from build123d import *

# Parameters (mm, degrees)
SKETCH1_W           = 71.75
SKETCH1_H           = 71.75
SKETCH1_R           = 4
BOSS_EXTRUDE1_DEPTH = 10
FILLET1_R           = 5
FILLET2_R           = 1
FILLET4_R           = 0.15
SKETCH2_R           = 1.525
CUT_EXTRUDE1_DEPTH  = 10


with BuildPart() as part:
    # Sketch1 → Boss-Extrude1 (new body)
    with BuildSketch(Plane.XY):
        Rectangle(SKETCH1_W, SKETCH1_H)
        with Locations((-29.125, 29.125)):
            Circle(SKETCH1_R, mode=Mode.SUBTRACT)
        with Locations((28.875, 29.125)):
            Circle(SKETCH1_R, mode=Mode.SUBTRACT)
        with Locations((28.875, -28.875)):
            Circle(SKETCH1_R, mode=Mode.SUBTRACT)
        with Locations((-29.125, -28.875)):
            Circle(SKETCH1_R, mode=Mode.SUBTRACT)
    extrude(amount=BOSS_EXTRUDE1_DEPTH)

    # Fillet1
    fillet1_edges = [part.edges().sort_by_distance(p)[0] for p in [
        (-35.875, 35.875, 5),
        (35.875, 35.875, 5),
        (35.875, -35.875, 5),
        (-35.875, -35.875, 5),
    ]]
    fillet(fillet1_edges, radius=FILLET1_R)

    # Fillet2
    fillet2_edges = [part.edges().sort_by_distance(p)[0] for p in [
        (35.875, 0, 10),
        (0, -35.875, 10),
        (-35.875, 0, 10),
        (0, 35.875, 10),
        (-34.410533906, 34.410533906, 10),
        (34.410533906, 34.410533906, 10),
        (-34.410533906, -34.410533906, 10),
        (34.410533906, -34.410533906, 10),
    ]]
    fillet(fillet2_edges, radius=FILLET2_R)

    # Fillet4
    fillet4_edges = [part.edges().sort_by_distance(p)[0] for p in [
        (-33.125, 29.125, 10),
        (24.875, 29.125, 10),
        (24.875, -28.875, 10),
        (-33.125, -28.875, 10),
    ]]
    fillet(fillet4_edges, radius=FILLET4_R)

    # Sketch2 → Cut-Extrude1 (cut)
    with BuildSketch(Plane.XY.offset(10)):
        with Locations((0, 22.5)):
            Circle(SKETCH2_R)
        with Locations((22.5, 0)):
            Circle(SKETCH2_R)
        with Locations((0, -22.5)):
            Circle(SKETCH2_R)
        with Locations((-22.5, 0)):
            Circle(SKETCH2_R)
    extrude(amount=-CUT_EXTRUDE1_DEPTH, mode=Mode.SUBTRACT)


solid = part.part
Model file for the job. Use its own axes, mm. Give positions to 0.01 mm unless a question says otherwise; leave off trailing zeros. Loops run counter-clockwise (first coordinate to the right, second up) from the corner with the lowest first, then second, coordinate; pieces in that order, holes last.
1) Wall check: line 1 (Y direction, x = 30, z = 4.5) (3 decimals); line 2 (Y direction, x = -22.5, z = 4.25) (3 decimals); line 3 (Y direction, x = 32.5, z = 1.75). Give the ranges that are in metal, low to high.
2) Saw through at C-C (y = -22.5). Write the cut outline in (x, z) (3 decimals).
3) Flat gauge pin, fed straight in: pin 1 Ø5 at (x, y) = (-29.125, -28.875) entering from +Z. Where does the tip first touch, or does it go through?
4) Pull direction Y, two halves, no side cores. Call faces 1 (the flat face through (0, 35.875, 4)), 2 (the cylindrical face through (28.35, -24.91, 4.86)), 3 (the flat face through (0, -35.875, 4)): +Y half, -Y half, draft (parallel to the pull), parting line (faces both ways), or undercut.
5) Saw through at A-A (x = 0). Write the cut outline in (y, z) (3 decimals), plus the area to 3 significant figures.
Answer block:
1. line 1: y = -35.875 to -32.714, -25.036 to 25.286, 32.964 to 35.875
1. line 2: y = -35.875 to -1.525, 1.525 to 35.875
1. line 3: y = -35.6 to -30.57, -27.18 to 27.43, 30.82 to 35.6
2. outline: (-35.875, 0) - (-1.525, 0) - (-1.525, 10) - (-34.875, 10) arc R1 ccw to (-35.875, 9) - close; (1.525, 0) - (35.875, 0) - (35.875, 9) arc R1 ccw to (34.875, 10) - (1.525, 10) - close
3. pin 1: passes through
4. face 1: +Y half
4. face 2: undercut
4. face 3: -Y half
5. outline: (-35.875, 0) - (-24.025, 0) - (-24.025, 10) - (-34.875, 10) arc R1 ccw to (-35.875, 9) - close; (-20.975, 0) - (20.975, 0) - (20.975, 10) - (-20.975, 10) - close; (24.025, 0) - (35.875, 0) - (35.875, 9) arc R1 ccw to (34.875, 10) - (24.025, 10) - close
5. area: 656 mm2
